Build history of the part. All positions in model axes, mm. Face numbers are marked on the shaded views. A direction names the side the tool comes from. Round coordinates to 2 decimals unless told otherwise and drop trailing zeros. Write each loop counter-clockwise with the first axis right and the second up, starting at its lowest first coordinate (ties: lowest second). Pieces come first, ordered by that corner, then holes. Notation, with made-up numbers: (-31.75, -31) - (-15.75, -31) arc R12 cw to (-15.75, -13) - close; hole circle Ø2 at (71, -29). An arc over 180 degrees is marked (long way). Answer as a JSON object with one key per item and string values. Group by question number.
Item 1: Two-plate mould, pull along Z, no slides. Class the marked faces 1, 2 and 3: +Z half, -Z half, draft (parallel to the pull), parting line (faces both ways), or undercut.
Item 2: Slice it at A-A, the plane x = -9. List the corners of the cut face in (y, z).
Item 3: Slice it at D-D, the plane x = 29.5. List the corners of the cut face in (y, z), then the cut area to 3 significant figures.
Item 4: Probe line 1 (Y direction, x = 30.5, z = 20.5); line 2 (X direction, y = 17, z = -8); line 3 (Z direction, x = 68, y = 8). List the from-to ranges inside material, lowest first. Write a range as from..to.
Item 5: Slice it at B-B, the plane y = 14. List the corners of the cut face in (x, z).
Item 6: Slice it at C-C, the plane z = 0. List the corners of the cut face in (x, y), then the cut area to 3 significant figures.
Item 7: Flat gauge pins, fed straight in: pin 1 (8 mm diameter, centred on x = -37.5, z = -1, fed in from +Y); pin 2 (3 mm diameter, centred on x = 5.5, y = 22.5, fed in from -Z); pin 3 (16 mm diameter, centred on x = -44.5, y = 11.5, fed in from -Z). Where does each tip first touch, or does it go through?
Item 8: Which spindle directions (+Z, -Z, +X, -X, +Y, -Y) get a long thin tool onto all of the face, cutting with end or side? Do the marked faces 4, 5, 6 and 7. Say none if no direction does.
from build123d import *

# Parameters (mm, degrees)
HUB_PROFILE_65_45_R   = 32.5
HUB_PROFILE_65_45_R_2 = 22.5
HUB_65_BORE_45_DEPTH  = 40
FORK_ARM_DEPTH        = 20
REAR_BLOCK_DEPTH      = 20


with BuildPart() as part:
    # Hub Profile Ø65-Ø45 → Hub Ø65 Bore Ø45 (new body)
    with BuildSketch(Plane(origin=(0, 0, 0), x_dir=(1, 0, 0), z_dir=(0, 1, 0))):
        with Locations(Location((0, 0, 0), (0, 0, 270))):
            Circle(HUB_PROFILE_65_45_R)
        with Locations(Location((0, 0, 0), (0, 0, 270))):
            Circle(HUB_PROFILE_65_45_R_2, mode=Mode.SUBTRACT)
    extrude(amount=HUB_65_BORE_45_DEPTH)

    # Fork Arm Profile → Fork Arm (add)
    with BuildSketch(Plane(origin=(0, 0, 0), x_dir=(1, 0, 0), z_dir=(0, 1, 0))):
        with BuildLine():
            Line((68, 6.576589216), (100, 6.576589216))
            Line((100, 6.576589216), (100, 13.210293464))
            ThreePointArc((100, 13.210293464), (98.79478546, 16.465996662), (95.760158675, 18.152171527))
            Line((95.760158675, 18.152171527), (5.067811416, 32.102449867))
            ThreePointArc((5.067811416, 32.102449867), (32.5, 0), (5.067811416, -32.102449867))
            Line((5.067811416, -32.102449867), (95.760158675, -18.152171527))
            ThreePointArc((95.760158675, -18.152171527), (98.79478546, -16.465996662), (100, -13.210293464))
            Line((100, -13.210293464), (100, -6.576589216))
            Line((100, -6.576589216), (68, -6.576589216))
            ThreePointArc((68, -6.576589216), (61.423410784, 0), (68, 6.576589216))
        make_face()
    extrude(amount=FORK_ARM_DEPTH)

    # Rear Block Profile 30x55 → Rear Block (add)
    with BuildSketch(Plane(origin=(0, 0, 0), x_dir=(1, 0, 0), z_dir=(0, 1, 0))):
        with BuildLine():
            Line((-55, -15), (-55, 15))
            Line((-55, 15), (-28.831406487, 15))
            ThreePointArc((-28.831406487, 15), (-32.5, 0), (-28.831406487, -15))
            Line((-28.831406487, -15), (-55, -15))
        make_face()
    extrude(amount=REAR_BLOCK_DEPTH)


solid = part.part
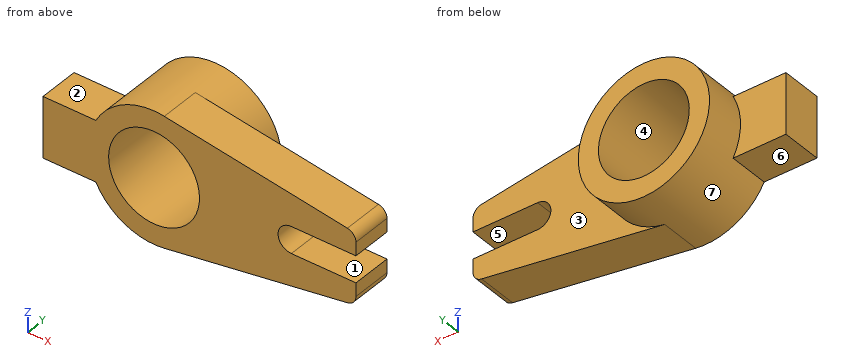
Geometry says:
{
 "1": {"face 1": "undercut", "face 2": "+Z half", "face 3": "draft"},
 "2": {"outline": "(0, -31.23) - (40, -31.23) - (40, -20.62) - (0, -20.62) - close; (0, 20.62) - (40, 20.62) - (40, 31.23) - (0, 31.23) - close"},
 "3": {"outline": "(0, -28.34) - (20, -28.34) - (20, -13.64) - (40, -13.64) - (40, 13.64) - (20, 13.64) - (20, 28.34) - (0, 28.34) - close", "area": "1,680 mm^2"},
 "4": {"line 1": "y = 0..20", "line 2": "x = -55..-21.03, 21.03..100", "line 3": "z = -22.42..-6.58, 6.58..22.42"},
 "5": {"outline": "(-55, -15) - (-28.83, -15) arc R32.5 ccw to (5.07, -32.1) - (95.76, -18.15) arc R5 ccw to (100, -13.21) - (100, -6.58) - (68, -6.58) arc R6.58 cw to (68, 6.58) - (100, 6.58) - (100, 13.21) arc R5 ccw to (95.76, 18.15) - (5.07, 32.1) arc R32.5 ccw to (-28.83, 15) - (-55, 15) - close; hole circle Ø45 at (0, 0)"},
 "6": {"outline": "(-55, 0) - (-22.5, 0) - (-22.5, 40) - (-32.5, 40) - (-32.5, 20) - (-55, 20) - close; (22.5, 0) - (61.42, 0) - (61.42, 20) - (32.5, 20) - (32.5, 40) - (22.5, 40) - close", "area": "1,830 mm^2"},
 "7": {"pin 1": "stops at y = 20", "pin 2": "stops at z = -32.25", "pin 3": "stops at z = -15"},
 "8": {"face 4": "+Y, -Y", "face 5": "+X, +Y, -Y", "face 6": "-Z, -X, +Y, -Y", "face 7": "+Y"}
}
